Input: dimensioned drawing with shaded views. Units: mm. Origin: part minimum x, y, z. A direction names the side the tool comes from. Round coordinates to 2 decimals unless told otherwise and drop trailing zeros. Loops run counter-clockwise (first coordinate to the right, second up) from the corner with the lowest first, then second, coordinate; pieces in that order, holes last. Notation, with made-up numbers: M -3.75,-15.75 L 18.25,-15.75 A19 cw 18.25,11.25 Z; hole C -5,9 d3. An arc over 180 degrees is marked long. Answer as a JSON object with one key per item and string values.
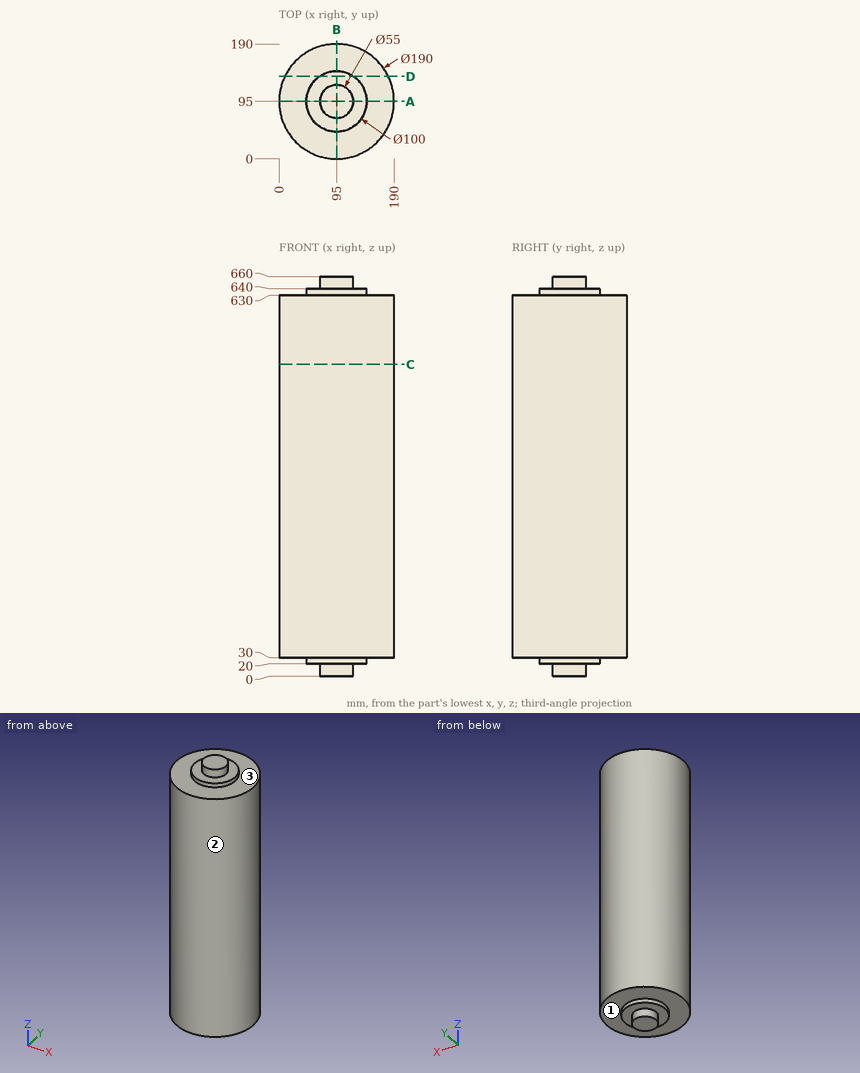
Item 1: Section D-D on y = 136.5. Return the cut outline in (x, z), then the cut area to 3 significant figures.
Answer sheet:
{"outline": "M 9.54,30 L 67.11,30 L 67.11,20 L 122.89,20 L 122.89,30 L 180.46,30 L 180.46,630 L 122.89,630 L 122.89,640 L 67.11,640 L 67.11,630 L 9.54,630 Z", "area": "104,000 mm²"}
Item 2: Line query: probe 1 along Z at (x, y) = (118, 148); probe 2 along Z at (x, y) = (57, 119.5); probe 3 along Y at (x, z) = (167.5, 524). Output: solid intervals per line, ascending. Write a range as from..to.
Answer sheet:
{"probe 1": "z = 30..630", "probe 2": "z = 20..640", "probe 3": "y = 33.61..156.39"}
Item 3: Section A-A on y = 95. Return the cut outline in (x, z), then the cut area to 3 significant figures.
Answer sheet:
{"outline": "M 0,30 L 45,30 L 45,20 L 67.5,20 L 67.5,0 L 122.5,0 L 122.5,20 L 145,20 L 145,30 L 190,30 L 190,630 L 145,630 L 145,640 L 122.5,640 L 122.5,660 L 67.5,660 L 67.5,640 L 45,640 L 45,630 L 0,630 Z", "area": "118,000 mm²"}
Item 4: Contact query for flat-ended pins moving along their axis: pin 1 Ø12 at (x, y) = (75, 65) entering from -Z; pin 2 Ø5 at (x, z) = (162, 432.5) entering from -Y; pin 3 Ø8 at (x, z) = (47.5, 280) entering from -Y. Output: stop coordinate, or through.
Answer sheet:
{"pin 1": "stops at z = 20", "pin 2": "stops at y = 25.25", "pin 3": "stops at y = 10.54"}
Item 5: Section C-C on z = 515.5. Return the cut outline in (x, y), then the cut area to 3 significant figures.
Answer sheet:
{"outline": "C 95,95 d190", "area": "28,400 mm²"}
Item 6: Access query for the marked faces 1, 2 and 3. Directions: +Z, -Z, +X, -X, +Y, -Y. A direction counts if a zero-diameter tool reaches every point of the face in a straight line with its end or side. Return the directions, or none.
Answer sheet:
{"face 1": "-Z", "face 2": "+Z, -Z", "face 3": "+Z"}
